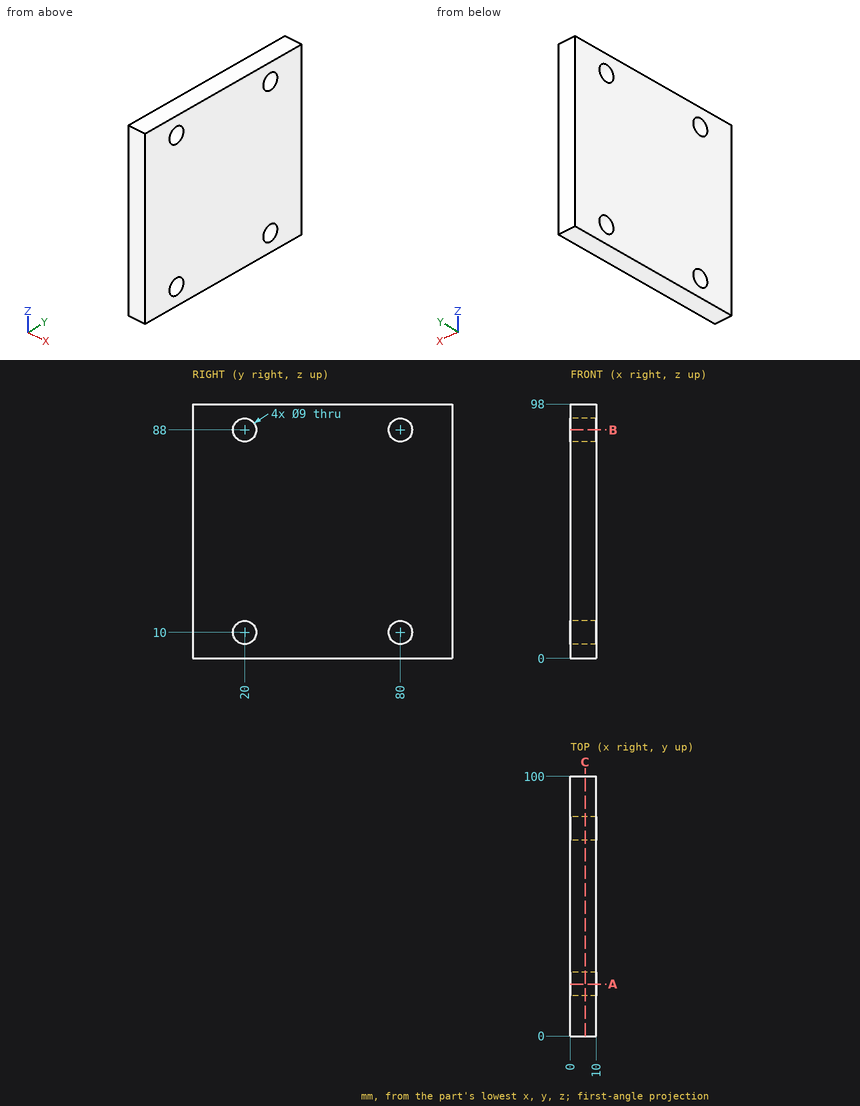
Geometry: see drawing. Coordinates: mm, zero at the bounding-box minimum. Coordinates: 2 decimals unless noted, no trailing zeros. Order: outer loops, then holes, each group sorted by start corner. A loop starts at its lowest first (then second) coordinate and runs counter-clockwise, first axis right, second up. Notation, with made-up numbers: M 62,62.25 L 77,62.25 A21 cw 77,79.25 Z; hole C 24,63.25 d5. An arc over 180 degrees is marked long. Answer as CSV lines item,"result".
1. Section A-A (y = 20). Return the cut outline in (x, z).
Reported:
outline,"M 0,0 L 10,0 L 10,5.5 L 0,5.5 Z; M 0,14.5 L 10,14.5 L 10,83.5 L 0,83.5 Z; M 0,92.5 L 10,92.5 L 10,98 L 0,98 Z"
2. Section C-C (x = 5.75). Return the cut outline in (y, z).
Reported:
outline,"M 0,0 L 100,0 L 100,98 L 0,98 Z; hole C 20,10 d9; hole C 20,88 d9; hole C 80,10 d9; hole C 80,88 d9"
3. First-contact query: P1, Ø4, axis at y = 71.5, z = 67.5, coming from the -X side; P2, Ø5.5, axis at y = 80, z = 88, coming from the -X side. Flat tips, straight axial feed; report the tip coordinate or a pass-through.
Reported:
P1,"x = 0"
P2,"through"
4. Section B-B (z = 88). Return the cut outline in (x, y), then the cut area to 3 significant figures.
Reported:
outline,"M 0,0 L 10,0 L 10,15.5 L 0,15.5 Z; M 0,24.5 L 10,24.5 L 10,75.5 L 0,75.5 Z; M 0,84.5 L 10,84.5 L 10,100 L 0,100 Z"
area,"820 mm2"
5. Material intervals for line 1 (Y direction, x = 4.5, z = 88), sorted ascending. Write a range as from..to.
Reported:
line 1,"0..15.5, 24.5..75.5, 84.5..100"
